For this review, take the finished solid that the model builds, in its own axes (mm). Coordinates: 2 decimals unless noted, no trailing zeros. Write each loop counter-clockwise with the first axis right and the second up, starting at its lowest first coordinate (ties: lowest second). Pieces come first, ordered by that corner, then holes.
```python
from build123d import *

# Parameters (mm, degrees)
SKETCH_1_W                = 120
SKETCH_1_H                = 16.4
EXTRUDE_1_DEPTH           = 3
SKETCH_2_R                = 1.65
SKETCH_2_R_2              = 1
CUT_EXTRUDE_2_DEPTH       = 2.3
SKETCH_3_R                = 1
CUT_EXTRUDE_3_DEPTH       = 61.854252111
SKETCH_4_W                = 0.35
SKETCH_4_H                = 5
CUT_EXTRUDE_5_DEPTH       = 121.317247309
CUT_EXTRUDE_6_DEPTH       = 61.653112039
CUT_EXTRUDE_7_DEPTH       = 61.854252111
CUT_EXTRUDE_7_DEPTH_BACK  = 61.854252111
SKETCH_7_R                = 1
CUT_EXTRUDE_10_DEPTH      = 61.854252111
CUT_EXTRUDE_10_DEPTH_BACK = 61.854252111
SKETCH_9_R                = 1


with BuildPart() as part:
    # 草图1 → 凸台-拉伸1 (new, symmetric)
    with BuildSketch(Plane.XY):
        Rectangle(SKETCH_1_W, SKETCH_1_H)
    extrude(amount=EXTRUDE_1_DEPTH, both=True)

    # 草图2 → 切除-拉伸2 (cut)
    # profile 1 of 4: a face of its own
    with BuildSketch(Plane.XY.offset(3)):
        with Locations((-10, 5.75)):
            Circle(SKETCH_2_R)
        with Locations((-10, 5.75)):
            Circle(SKETCH_2_R_2, mode=Mode.SUBTRACT)
    # profile 2 of 4: a face of its own
    with BuildSketch(Plane.XY.offset(3)):
        with Locations(Location((10, 5.75, 0), (0, 0, 180))):
            Circle(SKETCH_2_R)
        with Locations(Location((10, 5.75, 0), (0, 0, 180))):
            Circle(SKETCH_2_R_2, mode=Mode.SUBTRACT)
    # profile 3 of 4: a face of its own
    with BuildSketch(Plane.XY.offset(3)):
        with Locations((10, -5.75)):
            Circle(SKETCH_2_R)
        with Locations((10, -5.75)):
            Circle(SKETCH_2_R_2, mode=Mode.SUBTRACT)
    # profile 4 of 4: a face of its own
    with BuildSketch(Plane.XY.offset(3)):
        with Locations(Location((-10, -5.75, 0), (0, 0, 180))):
            Circle(SKETCH_2_R)
        with Locations(Location((-10, -5.75, 0), (0, 0, 180))):
            Circle(SKETCH_2_R_2, mode=Mode.SUBTRACT)
    extrude(amount=-CUT_EXTRUDE_2_DEPTH, mode=Mode.SUBTRACT)

    # 草图3 → 切除-拉伸3 (cut, through all)
    with BuildSketch(Plane.XY.offset(3)):
        with Locations((-10, 5.75)):
            Circle(SKETCH_3_R)
        with Locations((10, 5.75)):
            Circle(SKETCH_3_R)
        with Locations((-10, -5.75)):
            Circle(SKETCH_3_R)
        with Locations((10, -5.75)):
            Circle(SKETCH_3_R)
    extrude(amount=-CUT_EXTRUDE_3_DEPTH, mode=Mode.SUBTRACT)

    # 草图4 → 切除-拉伸5 (cut, through all)
    with BuildSketch(Plane.ZY.offset(60)):
        with Locations((-2.825, 0)):
            Rectangle(SKETCH_4_W, SKETCH_4_H)
        with BuildLine():
            Line((0.4, -2.5), (0.4, 2.5))
            Line((0.4, 2.5), (0.859619408, 2.959619408))
            ThreePointArc((0.859619408, 2.959619408), (1.702223965, 3.593279549), (2.345944084, 2.758335226))
            Line((2.345944084, 2.758335226), (2.65, 2.45427931))
            Line((2.65, 2.45427931), (3, 2.45427931))
            Line((3, 2.45427931), (3, -2.45427931))
            Line((3, -2.45427931), (2.65, -2.45427931))
            Line((2.65, -2.45427931), (2.345944084, -2.758335226))
            ThreePointArc((2.345944084, -2.758335226), (1.702223965, -3.593279549), (0.859619408, -2.959619408))
            Line((0.859619408, -2.959619408), (0.4, -2.5))
        make_face()
    extrude(amount=-CUT_EXTRUDE_5_DEPTH, mode=Mode.SUBTRACT)

    # 草图5 → 切除-拉伸6 (cut, through all)
    with BuildSketch(Plane.XY.offset(0.4)):
        with BuildLine():
            Line((-46, 1.7), (-22, 1.7))
            ThreePointArc((-22, 1.7), (-20.3, 0), (-22, -1.7))
            Line((-22, -1.7), (-46, -1.7))
            ThreePointArc((-46, -1.7), (-47.7, 0), (-46, 1.7))
        make_face()
        with BuildLine():
            Line((46, 1.7), (22, 1.7))
            ThreePointArc((22, 1.7), (20.3, 0), (22, -1.7))
            Line((22, -1.7), (46, -1.7))
            ThreePointArc((46, -1.7), (47.7, 0), (46, 1.7))
        make_face()
    extrude(amount=-CUT_EXTRUDE_6_DEPTH, mode=Mode.SUBTRACT)

    # 草图7 → 切除-拉伸7 (cut, two sides: drawn at the far end of the back side and taken through both)
    with BuildSketch(Plane(origin=(0, 0, -3), x_dir=(-1, 0, 0), z_dir=(0, 0, -1)).offset(-CUT_EXTRUDE_7_DEPTH_BACK)):
        with Locations((-58.249999998, -6)):
            Circle(SKETCH_7_R)
        with Locations((-58.249999998, 6)):
            Circle(SKETCH_7_R)
    extrude(amount=CUT_EXTRUDE_7_DEPTH + CUT_EXTRUDE_7_DEPTH_BACK, mode=Mode.SUBTRACT)

    # 草图9 → 切除-拉伸10 (cut, two sides: drawn at the far end of the back side and taken through both)
    with BuildSketch(Plane.XY.offset(3).offset(-CUT_EXTRUDE_10_DEPTH_BACK)):
        with Locations((-58.249989067, 5.99999379)):
            Circle(SKETCH_9_R)
        with Locations((-58.249989067, -6.00000621)):
            Circle(SKETCH_9_R)
    extrude(amount=CUT_EXTRUDE_10_DEPTH + CUT_EXTRUDE_10_DEPTH_BACK, mode=Mode.SUBTRACT)


solid = part.part
```
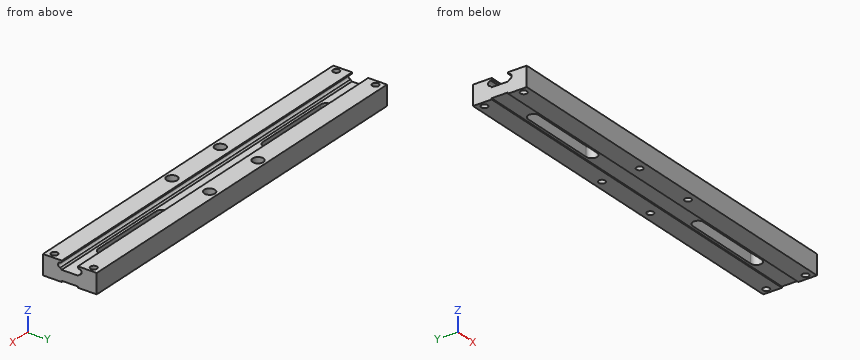
Q1. Add section C-C (x = -35.5). State the section outline as (y, z) points, then the cut area to 3 significant figures.
Ans:
outline: (-8.2, -3) - (-2.5, -3) - (-2.5, -2.65) - (-1.7, -2.65) - (-1.7, 0.4) - (-2.5, 0.4) - (-2.96, 0.86) arc R0.75 cw to (-2.76, 2.35) - (-2.45, 2.65) - (-2.45, 3) - (-8.2, 3) - close; (1.7, -2.65) - (2.5, -2.65) - (2.5, -3) - (8.2, -3) - (8.2, 3) - (2.45, 3) - (2.45, 2.65) - (2.76, 2.35) arc R0.75 cw to (2.96, 0.86) - (2.5, 0.4) - (1.7, 0.4) - close
area: 70.2 mm2
Q2. Add section B-B (y = 0). State the section outline as (x, z) points.
Ans:
outline: (-60, -2.65) - (-47.7, -2.65) - (-47.7, 0.4) - (-60, 0.4) - close; (-20.3, -2.65) - (20.3, -2.65) - (20.3, 0.4) - (-20.3, 0.4) - close; (47.7, -2.65) - (60, -2.65) - (60, 0.4) - (47.7, 0.4) - close
Q3. Clearance check with a flat-ended pin moving along its axis: pin 1 Ø2.5 at (x, y) = (10, 5.75) entering from +Z. State where the tip first meets the part, or that it passes through.
Ans:
pin 1: stops at z = 0.7
Q4. Add section A-A (x = 10). Give the number of separate pieces and of enclosed holes in the cut face, then the cut area to 3 significant figures.
Ans:
separate pieces: 3
enclosed holes: 0
area: 50.6 mm2
Q5. For probe 1 along Y at (x, z) = (10, 1.5); probe 2 along X at (y, z) = (-5.25, -2.6); probe 3 along Y at (x, z) = (-31.5, -2.35), list the stretches that pass through material, from the lowest coordinate up.
Ans:
probe 1: y = -8.2 to -7.4, -4.1 to -3.59, 3.59 to 4.1, 7.4 to 8.2
probe 2: x = -60 to -58.91, -57.59 to -10.87, -9.13 to 9.13, 10.87 to 57.59, 58.91 to 60
probe 3: y = -8.2 to -1.7, 1.7 to 8.2
